Check sheet for the drawn part. Datum: minimum x, y, z corner. Units: mm. Give positions to 0.01 mm unless a question says otherwise; leave off trailing zeros. Order: outer loops, then holes, each group sorted by start corner. A loop starts at its lowest first (then second) coordinate and runs counter-clockwise, first axis right, second up.
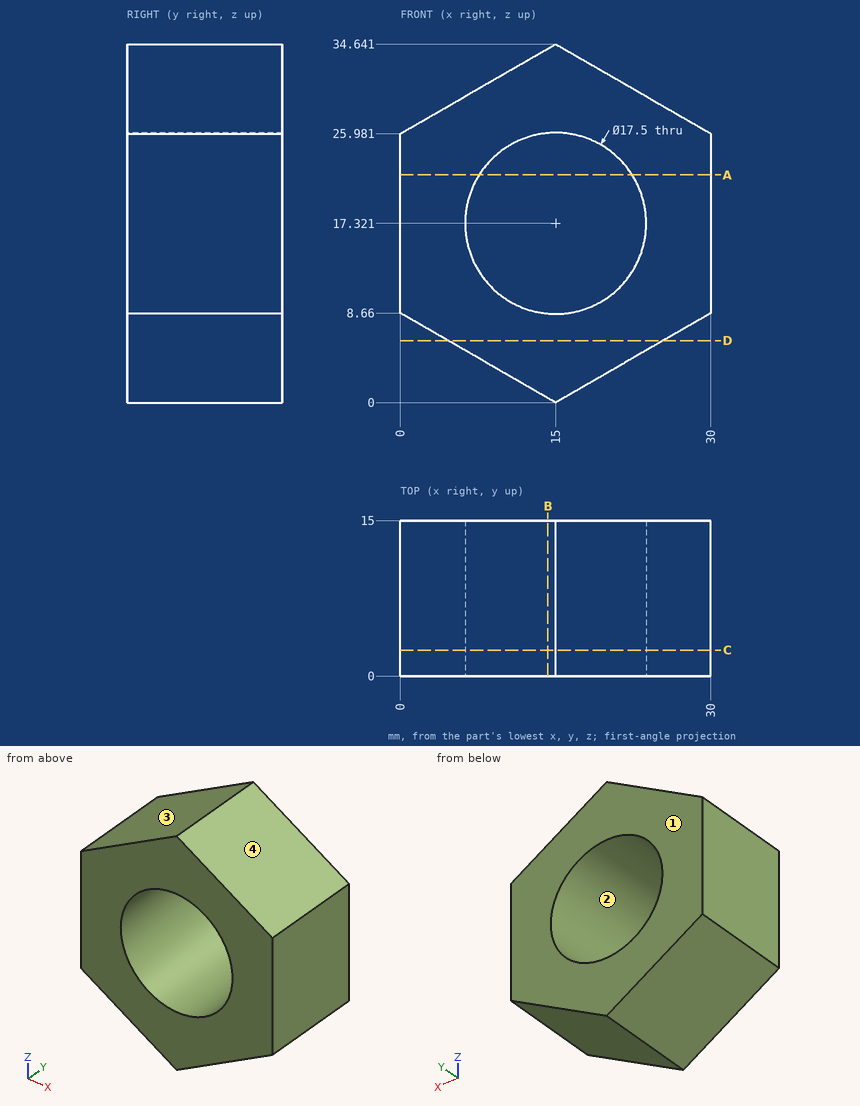
Item 1: Sectioned sample at B-B (x = 14.25). Enter the section's corners in (y, z), and give its area (3 significant figures).
Reported:
outline: (0, 0.43) - (15, 0.43) - (15, 8.6) - (0, 8.6) - close; (0, 26.04) - (15, 26.04) - (15, 34.21) - (0, 34.21) - close
area: 245 mm2
Item 2: Gauge pin test, flat ends, axial feed: pin 1 (4 mm diameter, centred on x = 7, y = 3, fed in from -Z) (1 decimal); pin 2 (5 mm diameter, centred on x = 8.5, y = 11.5, fed in from +Z); pin 3 (6 mm diameter, centred on x = 17.5, z = 10, fed in from +Y); pin 4 (14 mm diameter, centred on x = 15, z = 17.32, fed in from -Y). Record the tip position at first contact, or that the pin passes through.
Reported:
pin 1: stops at z = 3.5
pin 2: stops at z = 32.33
pin 3: stops at y = 15
pin 4: passes through
Item 3: Sectioned sample at A-A (z = 22). Enter the section's corners in (x, y), and give its area (3 significant figures).
Reported:
outline: (0, 0) - (7.61, 0) - (7.61, 15) - (0, 15) - close; (22.39, 0) - (30, 0) - (30, 15) - (22.39, 15) - close
area: 228 mm2
Item 4: Sectioned sample at D-D (z = 6). Enter the section's corners in (x, y), and give its area (3 significant figures).
Reported:
outline: (4.61, 0) - (25.39, 0) - (25.39, 15) - (4.61, 15) - close
area: 312 mm2
Item 5: Draft check along X on the marked faces 1, 2, 3 and 4. Enter one of: released by +X, released by -X, zero draft, split by the parting line, or undercut.
Reported:
face 1: zero draft
face 2: undercut
face 3: released by -X
face 4: released by +X
Item 6: Scan lines: L1, parallel to Z at x = 15, y = 7; L2, parallel to X at y = 1.5, z = 11.5 (1 decimal); L3, parallel to X at y = 9.75, z = 12.5. Record each from-to range of solid material in increasing order.
Reported:
L1: z = 0 to 8.57, 26.07 to 34.64
L2: x = 0 to 8.5, 21.5 to 30
L3: x = 0 to 7.7, 22.3 to 30
Item 7: Sectioned sample at C-C (y = 2.5). Enter the section's corners in (x, z).
Reported:
outline: (0, 8.66) - (15, 0) - (30, 8.66) - (30, 25.98) - (15, 34.64) - (0, 25.98) - close; hole circle Ø17.5 at (15, 17.32)
